from build123d import *

# Parameters (mm, degrees)
SKETCH1_W                 = 210
SKETCH1_H                 = 80
BOSS_EXTRUDE1_DEPTH       = 13
SKETCH2_R                 = 5
SKETCH2_R_2               = 3
CUT_EXTRUDE1_DEPTH        = 6
CUT_EXTRUDE2_REACH        = 115.111
SKETCH2_5_R               = 3
M6X1_0_TAPPED_HOLE1_D     = 5
M6X1_0_TAPPED_HOLE1_DEPTH = 15
M6X1_0_TAPPED_HOLE1_TIP   = 1.502151548
SKETCH8_R                 = 5
SKETCH8_R_2               = 3
CUT_EXTRUDE3_DEPTH        = 6
CUT_EXTRUDE4_REACH        = 115.111
SKETCH8_4_R               = 3
M6X1_0_TAPPED_HOLE2_D     = 5
M6X1_0_TAPPED_HOLE2_DEPTH = 15
M6X1_0_TAPPED_HOLE2_TIP   = 1.502151548


with BuildPart() as part:
    # Sketch1 → Boss-Extrude1 (new body)
    with BuildSketch(Plane.XY):
        Rectangle(SKETCH1_W, SKETCH1_H)
    extrude(amount=BOSS_EXTRUDE1_DEPTH)

    # Sketch2 → Cut-Extrude1 (cut)
    # profile 1 of 2: a face of its own
    with BuildSketch(Plane(origin=(0, 0, 0), x_dir=(-1, 0, 0), z_dir=(0, 0, -1))):
        with Locations((-38.524202037, 23.616817232)):
            Circle(SKETCH2_R)
        with Locations((-38.524202037, 23.616817232)):
            Circle(SKETCH2_R_2, mode=Mode.SUBTRACT)
    # profile 2 of 2: a face of its own
    with BuildSketch(Plane(origin=(0, 0, 0), x_dir=(-1, 0, 0), z_dir=(0, 0, -1))):
        with Locations((38.548404074, 23.616912244)):
            Circle(SKETCH2_R)
        with Locations((38.548404074, 23.616912244)):
            Circle(SKETCH2_R_2, mode=Mode.SUBTRACT)
    extrude(amount=-CUT_EXTRUDE1_DEPTH, mode=Mode.SUBTRACT)

    # Sketch2<5> → Cut-Extrude2 (cut, up to next)
    with BuildSketch(Plane(origin=(0, 0, 0), x_dir=(-1, 0, 0), z_dir=(0, 0, -1)), mode=Mode.PRIVATE) as cut_extrude2_sk1:
        with Locations((-38.524202037, 23.616817232)):
            Circle(SKETCH2_5_R)
    cut_extrude2_tool1 = extrude(cut_extrude2_sk1.sketch, amount=-CUT_EXTRUDE2_REACH, mode=Mode.PRIVATE) & part.part
    # Sketch2<5> → Cut-Extrude2 (cut, up to next)
    with BuildSketch(Plane(origin=(0, 0, 0), x_dir=(-1, 0, 0), z_dir=(0, 0, -1)), mode=Mode.PRIVATE) as cut_extrude2_sk2:
        with Locations((38.548404074, 23.616912244)):
            Circle(SKETCH2_5_R)
    cut_extrude2_tool2 = extrude(cut_extrude2_sk2.sketch, amount=-CUT_EXTRUDE2_REACH, mode=Mode.PRIVATE) & part.part
    add(cut_extrude2_tool1.solids().sort_by_distance((38.524202, 23.616817, 0))[0], mode=Mode.SUBTRACT)
    add(cut_extrude2_tool2.solids().sort_by_distance((-38.548404, 23.616912, 0))[0], mode=Mode.SUBTRACT)

    # M6x1.0 Tapped Hole1
    with Locations(Plane(origin=(105, -32.5, 6.5), x_dir=(0, 0, 1), z_dir=(1, 0, 0))):
        with Locations((0, 0)):
            Hole(M6X1_0_TAPPED_HOLE1_D / 2, depth=M6X1_0_TAPPED_HOLE1_DEPTH)
            with Locations((0, 0, -(M6X1_0_TAPPED_HOLE1_DEPTH + M6X1_0_TAPPED_HOLE1_TIP / 2))):  # 118° drill point
                Cone(0, M6X1_0_TAPPED_HOLE1_D / 2, M6X1_0_TAPPED_HOLE1_TIP, mode=Mode.SUBTRACT)

    # Sketch8 → Cut-Extrude3 (cut)
    # profile 1 of 3: a face of its own
    with BuildSketch(Plane(origin=(0, 0, 0), x_dir=(-1, 0, 0), z_dir=(0, 0, -1))):
        with Locations((-80, -32.5)):
            Circle(SKETCH8_R)
        with Locations((-80, -32.5)):
            Circle(SKETCH8_R_2, mode=Mode.SUBTRACT)
    # profile 2 of 3: a face of its own
    with BuildSketch(Plane(origin=(0, 0, 0), x_dir=(-1, 0, 0), z_dir=(0, 0, -1))):
        with Locations((80, -32.5)):
            Circle(SKETCH8_R)
        with Locations((80, -32.5)):
            Circle(SKETCH8_R_2, mode=Mode.SUBTRACT)
    # profile 3 of 3: a face of its own
    with BuildSketch(Plane(origin=(0, 0, 0), x_dir=(-1, 0, 0), z_dir=(0, 0, -1))):
        with Locations((0, -32.5)):
            Circle(SKETCH8_R)
        with Locations((0, -32.5)):
            Circle(SKETCH8_R_2, mode=Mode.SUBTRACT)
    extrude(amount=-CUT_EXTRUDE3_DEPTH, mode=Mode.SUBTRACT)

    # Sketch8<4> → Cut-Extrude4 (cut, up to next)
    with BuildSketch(Plane(origin=(0, 0, 0), x_dir=(-1, 0, 0), z_dir=(0, 0, -1)), mode=Mode.PRIVATE) as cut_extrude4_sk1:
        with Locations((-80, -32.5)):
            Circle(SKETCH8_4_R)
    cut_extrude4_tool1 = extrude(cut_extrude4_sk1.sketch, amount=-CUT_EXTRUDE4_REACH, mode=Mode.PRIVATE) & part.part
    # Sketch8<4> → Cut-Extrude4 (cut, up to next)
    with BuildSketch(Plane(origin=(0, 0, 0), x_dir=(-1, 0, 0), z_dir=(0, 0, -1)), mode=Mode.PRIVATE) as cut_extrude4_sk2:
        with Locations((0, -32.5)):
            Circle(SKETCH8_4_R)
    cut_extrude4_tool2 = extrude(cut_extrude4_sk2.sketch, amount=-CUT_EXTRUDE4_REACH, mode=Mode.PRIVATE) & part.part
    # Sketch8<4> → Cut-Extrude4 (cut, up to next)
    with BuildSketch(Plane(origin=(0, 0, 0), x_dir=(-1, 0, 0), z_dir=(0, 0, -1)), mode=Mode.PRIVATE) as cut_extrude4_sk3:
        with Locations((80, -32.5)):
            Circle(SKETCH8_4_R)
    cut_extrude4_tool3 = extrude(cut_extrude4_sk3.sketch, amount=-CUT_EXTRUDE4_REACH, mode=Mode.PRIVATE) & part.part
    add(cut_extrude4_tool1.solids().sort_by_distance((80, -32.5, 0))[0], mode=Mode.SUBTRACT)
    add(cut_extrude4_tool2.solids().sort_by_distance((0, -32.5, 0))[0], mode=Mode.SUBTRACT)
    add(cut_extrude4_tool3.solids().sort_by_distance((-80, -32.5, 0))[0], mode=Mode.SUBTRACT)

    # M6x1.0 Tapped Hole2
    with Locations(Plane(origin=(105, 28, 6.5), x_dir=(0, 0, 1), z_dir=(1, 0, 0))):
        with Locations((0, 0)):
            Hole(M6X1_0_TAPPED_HOLE2_D / 2, depth=M6X1_0_TAPPED_HOLE2_DEPTH)
            with Locations((0, 0, -(M6X1_0_TAPPED_HOLE2_DEPTH + M6X1_0_TAPPED_HOLE2_TIP / 2))):  # 118° drill point
                Cone(0, M6X1_0_TAPPED_HOLE2_D / 2, M6X1_0_TAPPED_HOLE2_TIP, mode=Mode.SUBTRACT)


solid = part.part
Could you check a few things on this model? Use its own coordinates, in mm. A direction names the side the tool comes from. Round coordinates to 2 decimals unless told otherwise and drop trailing zeros. Write each loop counter-clockwise with the first axis right and the second up, starting at its lowest first coordinate (ties: lowest second). Pieces come first, ordered by that corner, then holes. Notation, with made-up numbers: (46.25, 19.25) - (63.25, 19.25) arc R26 cw to (63.25, 36.25) - close; hole circle Ø2 at (-18, 67.5). An arc over 180 degrees is marked (long way). Put each result on its own line as item: value. Start each with the question number.
(1) Thinking about a two-plate mould opening in Z: for faces 1 (the flat face through (-41, 21, 6)), 2 (the conical face through (88.76, -32.11, 6.7)), 3 (the cylindrical face through (97, 26, 5)), 4 (the cylindrical face through (83, -32.4, 9.5)), which applies, released by +Z, released by -Z, zero draft, split by the parting line, or undercut?
(2) For faces 5 (the cylindrical face through (97.4, -34.61, 5.16)), 6 (the flat face through (-82, -35, 6)), 7 (the cylindrical face through (41.52, 23.75, 9.45)), which set-ups out of +Z, -Z, +X, -X, +Y, -Y let a thin tool reach every point of the face, with its end or its side?
(3) Will this pin go through, and if not, where does the flat tip stop? pin 1 (3 mm diameter, centred on x = 1, y = -30.5, fed in from -Z).
(4) I need wall thicknesses on probe 1 along Y at (x, z) = (0, 10.75); probe 2 along Z at (x, y) = (99, -32.5); probe 3 along Y at (x, z) = (94, 6.5). Which ranges of each line are inside material? Lowest first, please.
(5) I want a section at A-A, the plane x = 0. Please give me the cut outline in (y, z).
Here are the results:
1. face 1: released by -Z
1. face 2: undercut
1. face 3: undercut
1. face 4: zero draft
2. face 5: +X
2. face 6: -Z
2. face 7: +Z, -Z
3. pin 1: stops at z = 6
4. probe 1: y = -40 to -35.5, -29.5 to 40
4. probe 2: z = 0 to 4, 9 to 13
4. probe 3: y = -40 to -35, -30 to 25.5, 30.5 to 40
5. outline: (-40, 0) - (-37.5, 0) - (-37.5, 6) - (-35.5, 6) - (-35.5, 13) - (-40, 13) - close; (-29.5, 6) - (-27.5, 6) - (-27.5, 0) - (40, 0) - (40, 13) - (-29.5, 13) - close
